Could you check a few things on this model? Use its own coordinates, in mm. A direction names the side the tool comes from. Coordinates: 2 decimals unless noted, no trailing zeros. Loops run counter-clockwise (first coordinate to the right, second up) from the corner with the lowest first, then second, coordinate; pieces in that order, holes last.
from build123d import *

# Parameters (mm, degrees)
SKETCH_1_W          = 25
SKETCH_1_H          = 120
EXTRUDE_1_DEPTH     = 10
SKETCH_2_R          = 8
CUT_EXTRUDE_1_DEPTH = 2
CUT_EXTRUDE_2_REACH = 64.099
SKETCH_3_R          = 8.5


with BuildPart() as part:
    # 草图1 → 凸台-拉伸1 (new body)
    with BuildSketch(Plane(origin=(0, 0, 0), x_dir=(1, 0, 0), z_dir=(0, 1, 0))):
        Rectangle(SKETCH_1_W, SKETCH_1_H)
    extrude(amount=EXTRUDE_1_DEPTH)

    # 草图2 → 切除-拉伸1 (cut)
    with BuildSketch(Plane(origin=(0, 10, 0), x_dir=(1, 0, 0), z_dir=(0, 1, 0))):
        with Locations(Location((0, 46, 0), (0, 0, 270))):
            Circle(SKETCH_2_R)
        with Locations(Location((0, -46, 0), (0, 0, 270))):
            Circle(SKETCH_2_R)
    extrude(amount=-CUT_EXTRUDE_1_DEPTH, mode=Mode.SUBTRACT)

    # 草图3 → 切除-拉伸2 (cut, up to next)
    with BuildSketch(Plane(origin=(0, 10, 0), x_dir=(1, 0, 0), z_dir=(0, 1, 0)), mode=Mode.PRIVATE) as cut_extrude_2_sk1:
        with Locations(Location((0, 0, 0), (0, 0, 270))):
            Circle(SKETCH_3_R)
    cut_extrude_2_tool1 = extrude(cut_extrude_2_sk1.sketch, amount=-CUT_EXTRUDE_2_REACH, mode=Mode.PRIVATE) & part.part
    add(cut_extrude_2_tool1.solids().sort_by_distance((0, 10, 0))[0], mode=Mode.SUBTRACT)


solid = part.part
(1) Imagine slicing it at A-A, the plane z = 0. Write out the boundary of the cut face in (x, y).
Answers:
outline: (-12.5, 0) - (-8.5, 0) - (-8.5, 10) - (-12.5, 10) - close; (8.5, 0) - (12.5, 0) - (12.5, 10) - (8.5, 10) - close
(2) We'd pull the mould along Z, two halves only. Please class faces 3 (the face through (12.5, 5, 1)), 4 (the face through (0, 5, 60)), 5 (the face through (8.428, 5.07, -1.107)), 6 (the face through (0, 8, -46)): +Z half, -Z half, draft (parallel to the pull), parting line (faces both ways), or undercut.
Answers:
face 3: draft
face 4: +Z half
face 5: undercut
face 6: undercut
(3) For pin 1 (14.5 mm diameter, centred on x = 0, z = -46, fed in from -Y); pin 2 (5 mm diameter, centred on x = -0.5, z = -43, fed in from +Y); pin 3 (10 mm diameter, centred on x = 0, z = 0, fed in from +Y), each with a flat end and sliding along its axis, tell me the tip position at first contact or that it passes through.
Answers:
pin 1: stops at y = 0
pin 2: stops at y = 8
pin 3: passes through
(4) Imagine slicing it at B-B, the plane x = 0. Write out the boundary of the cut face in (y, z), and give its area (3 significant figures).
Answers:
outline: (0, -60) - (10, -60) - (10, -54) - (8, -54) - (8, -38) - (10, -38) - (10, -8.5) - (0, -8.5) - close; (0, 8.5) - (10, 8.5) - (10, 38) - (8, 38) - (8, 54) - (10, 54) - (10, 60) - (0, 60) - close
area: 966 mm2
(5) I need wall thicknesses on probe 1 along Z at (x, y) = (4.75, 8.5); probe 2 along X at (y, z) = (9.05, -46); probe 3 along X at (y, z) = (6, 0). Which ranges of each line are inside material? Lowest first, please.
Answers:
probe 1: z = -60 to -52.44, -39.56 to -7.05, 7.05 to 39.56, 52.44 to 60
probe 2: x = -12.5 to -8, 8 to 12.5
probe 3: x = -12.5 to -8.5, 8.5 to 12.5
(6) Imagine slicing it at C-C, the plane y = 3. Write out the boundary of the cut face in (x, z).
Answers:
outline: (-12.5, -60) - (12.5, -60) - (12.5, 60) - (-12.5, 60) - close; hole circle Ø17 at (0, 0)
(7) Imagine slicing it at D-D, the plane z = 46. Write out the boundary of the cut face in (x, y).
Answers:
outline: (-12.5, 0) - (12.5, 0) - (12.5, 10) - (8, 10) - (8, 8) - (-8, 8) - (-8, 10) - (-12.5, 10) - close
(8) Which directions (+Z, -Z, +X, -X, +Y, -Y) give clear straight access to the entire face, cutting with the end or side of a thin tool? Please do faces 1 (the face through (-4.868, 9.014, 39.651)), 2 (the face through (-12.5, 5, 1)).
Answers:
face 1: +Y
face 2: +Z, -Z, -X, +Y, -Y
